from build123d import *

# Parameters (mm, degrees)
SKETCH_1_W      = 50
SKETCH_1_H      = 50
SKETCH_1_R      = 5
EXTRUDE_1_DEPTH = 10


with BuildPart() as part:
    # 草图1 → 凸台-拉伸1 (new body)
    with BuildSketch(Plane.XY):
        with Locations((25, 25)):
            Rectangle(SKETCH_1_W, SKETCH_1_H)
        with Locations((25, 25)):
            Circle(SKETCH_1_R, mode=Mode.SUBTRACT)
    extrude(amount=EXTRUDE_1_DEPTH)


solid = part.part
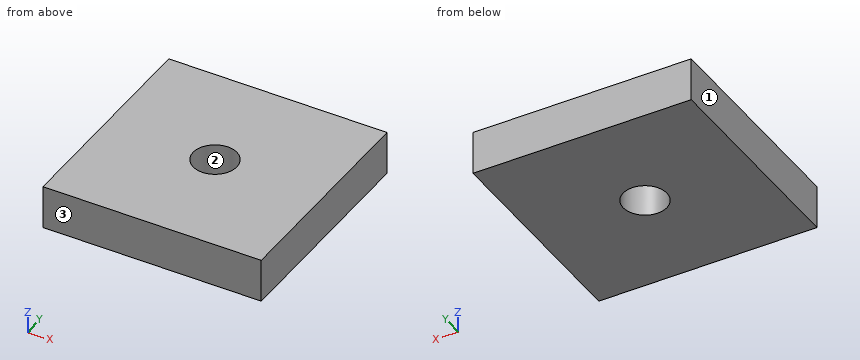
Source: CAD feature listing. Evaluate the final solid. Frame: model axes, mm. Face numbers are marked on the shaded views. Round coordinates to 2 decimals unless told otherwise and drop trailing zeros. Order: outer loops, then holes, each group sorted by start corner. A loop starts at its lowest first (then second) coordinate and runs counter-clockwise, first axis right, second up. Notation, with made-up numbers: (-6, -21) - (43, -21) arc R18 cw to (43, -15) - close; hole circle Ø5 at (-33.75, -30). An arc over 180 degrees is marked (long way). Use a Markdown table: item, result. Add a question column.
1. First-contact query: pin 1 (8 mm diameter, centred on x = 25, y = 25, fed in from +Z). Flat tip, straight axial feed; report the tip coordinate or a pass-through.
2. Section query A-A (x = 25). Return the cut outline in (y, z), then the cut area to 3 significant figures.
3. Mould query, pull axis Y, two halves, no side actions, for the marked faces 1, 2 and 3. Classes: +Y half, -Y half, draft (parallel to the pull), parting line (faces both ways), or undercut.
4. Section query C-C (z = 4). Return the cut outline in (x, y), then the cut area to 3 significant figures.
5. Line query: probe 1 along Y at (x, z) = (25, 3.5); probe 2 along Y at (x, z) = (26, 4.75); probe 3 along X at (y, z) = (25.5, 2.5). Output: solid intervals per line, ascending.
Derived:
| question | item | result |
|---|---|---|
| 1 | pin 1 | through |
| 2 | outline | (0, 0) - (20, 0) - (20, 10) - (0, 10) - close; (30, 0) - (50, 0) - (50, 10) - (30, 10) - close |
| 2 | area | 400 mm2 |
| 3 | face 1 | draft |
| 3 | face 2 | undercut |
| 3 | face 3 | -Y half |
| 4 | outline | (0, 0) - (50, 0) - (50, 50) - (0, 50) - close; hole circle Ø10 at (25, 25) |
| 4 | area | 2,420 mm2 |
| 5 | probe 1 | 0 to 20, 30 to 50 |
| 5 | probe 2 | 0 to 20.1, 29.9 to 50 |
| 5 | probe 3 | 0 to 20.03, 29.97 to 50 |
